Read the model definition and answer for the solid it produces. Units are mm, in the model's axes. Coordinates: 2 decimals unless noted, no trailing zeros. Loops run counter-clockwise (first coordinate to the right, second up) from the corner with the lowest first, then second, coordinate; pieces in that order, holes last. Notation, with made-up numbers: (71.25, 33.25) - (124.25, 33.25) arc R25 ccw to (124.25, 69.25) - close; hole circle Ø11 at (18, 25). An arc over 180 degrees is marked (long way). Use one line per item in the form item = value. Start each with the question number.
1) Consider line 1 (X direction, y = 7.5, z = 10.5); line 2 (Z direction, x = 3, y = 5.5); line 3 (Z direction, x = 40.5, y = 3.25). Determine where each line is inside the solid, lowest interval first.
2) Each of these flat-tipped pins is pushed along its axis until it touches: P1, Ø5, axis at y = 5, z = 12.34, coming from the -X side; P2, Ø5, axis at x = -5, y = 7.5, coming from the +Z side; P3, Ø3, axis at y = 5, z = 12.34, coming from the +X side; P4, Ø5, axis at y = 4, z = -44, coming from the -X side. Where does it stop, or does it pass through?
3) A cutting plane is placed at A-A (z = 30). Give the vertices of the cut face in (x, y).
4) A cutting plane is placed at C-C (y = 5). State how many separate pieces and enclosed holes the cut face has, and give its area (3 significant figures).
5) A cutting plane is placed at D-D (x = 32.5). Give the vertices of the cut face in (y, z), and give its area (3 significant figures).
6) A cutting plane is placed at B-B (x = 4.5). Give the vertices of the cut face in (y, z), and give its area (3 significant figures).
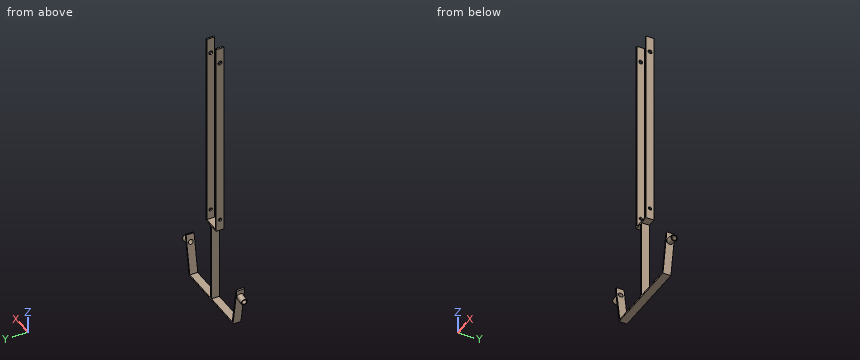
from build123d import *

# Parameters (mm, degrees)
EXTRUDE_1_DEPTH     = 10
SKETCH_3_W          = 100
SKETCH_3_H          = 10
EXTRUDE_2_DEPTH     = 1
EXTRUDE_3_DEPTH     = 10
SKETCH_6_R          = 4
SKETCH_6_R_2        = 3
EXTRUDE_4_DEPTH     = 10
CUT_EXTRUDE_START   = -20
SKETCH_7_R          = 3
CUT_EXTRUDE_1_DEPTH = 20
SKETCH_9_R          = 2.5
CUT_EXTRUDE_2_DEPTH = 274
SKETCH_10_R         = 2
CUT_EXTRUDE_3_DEPTH = 45


with BuildPart() as part:
    # 草图1 → 凸台-拉伸1 (new body)
    with BuildSketch(Plane(origin=(0, 0, 0), x_dir=(1, 0, 0), z_dir=(0, 1, 0))):
        Polygon((-10, -248), (-10, 0), (10, 0), (10, -248), (12, -248), (12, 2), (-12, 2), (-12, -248), align=None)
    extrude(amount=EXTRUDE_1_DEPTH)

    # 草图3 → 凸台-拉伸2 (add, symmetric)
    with BuildSketch(Plane(origin=(0, 0, 0), x_dir=(0, 0, -1), z_dir=(1, 0, 0))):
        with Locations((52, 5)):
            Rectangle(SKETCH_3_W, SKETCH_3_H)
    extrude(amount=EXTRUDE_2_DEPTH, both=True)

    # 草图4 → 凸台-拉伸3 (add)
    with BuildSketch(Plane(origin=(0, 0, 0), x_dir=(1, 0, 0), z_dir=(0, 1, 0))):
        Polygon((-50, 102), (50, 102), (58.682408883, 52.759612349), (60.652024389, 53.106908705), (51.678199262, 104), (-51.678199262, 104), (-60.652024389, 53.106908705), (-58.682408883, 52.759612349), align=None)
    extrude(amount=EXTRUDE_3_DEPTH)

    # 草图6 → 凸台-拉伸4 (add)
    with BuildSketch(Plane(origin=(-67.904958335, 0, -11.973476278), x_dir=(-0.17364817766693408, 0, 0.9848077530122076), z_dir=(-0.9848077530122076, 0, -0.17364817766693408))):
        with Locations(Location((-51.767981924, 5, 0), (0, 0, 180))):
            Circle(SKETCH_6_R)
        with Locations((-51.767981924, 5)):
            Circle(SKETCH_6_R_2, mode=Mode.SUBTRACT)
    extrude_4 = extrude(amount=EXTRUDE_4_DEPTH)

    # 草图7 → 切除-拉伸1 (cut)
    with BuildSketch(Plane(origin=(-67.904958335, 0, -11.973476278), x_dir=(-0.17364817766693408, 0, 0.9848077530122076), z_dir=(-0.9848077530122076, 0, -0.17364817766693408)).offset(CUT_EXTRUDE_START)):
        with Locations((-51.767981924, 5)):
            Circle(SKETCH_7_R)
    cut_extrude_1 = extrude(amount=CUT_EXTRUDE_1_DEPTH, mode=Mode.SUBTRACT)

    # 镜向1: 凸台-拉伸4, 切除-拉伸1 across plane
    add(extrude_4.mirror(Plane(origin=(0, 0, 0), x_dir=(0, 0, 1), z_dir=(1, 0, 0))))
    add(cut_extrude_1.mirror(Plane(origin=(0, 0, 0), x_dir=(0, 0, 1), z_dir=(1, 0, 0))), mode=Mode.SUBTRACT)

    # 草图9 → 切除-拉伸2 (cut)
    with BuildSketch(Plane.ZY.offset(12)):
        with Locations((228, 5)):
            Circle(SKETCH_9_R)
    extrude(amount=-CUT_EXTRUDE_2_DEPTH, mode=Mode.SUBTRACT)

    # 草图10 → 切除-拉伸3 (cut)
    with BuildSketch(Plane.ZY.offset(12)):
        with Locations((12.339097651, 5)):
            Circle(SKETCH_10_R)
    extrude(amount=-CUT_EXTRUDE_3_DEPTH, mode=Mode.SUBTRACT)


solid = part.part
Found:
q1.line_1 = -12 to -10, 10 to 12
q1.line_2 = -104 to -102, -2 to 0
q1.line_3 = -104 to -102
q2.P1 = -12
q2.P2 = 0
q2.P3 = through
q2.P4 = -1
q3.outline = (-12, 0) - (-10, 0) - (-10, 10) - (-12, 10) - close; (10, 0) - (12, 0) - (12, 10) - (10, 10) - close
q4.separate_pieces = 7
q4.enclosed_holes = 0
q4.area = 1,630 mm^2
q5.outline = (0, -104) - (10, -104) - (10, -102) - (0, -102) - close
q5.area = 20.0 mm^2
q6.outline = (0, -104) - (10, -104) - (10, -102) - (0, -102) - close; (0, -2) - (10, -2) - (10, 0) - (0, 0) - close
q6.area = 40.0 mm^2
